Here's how the part is built. I have some questions about the finished solid (model axes, mm). A direction names the side the tool comes from. Coordinates: 2 decimals unless noted, no trailing zeros. Write each loop counter-clockwise with the first axis right and the second up, starting at its lowest first coordinate (ties: lowest second). Pieces come first, ordered by that corner, then holes. Notation, with made-up numbers: M 83.5,-31 L 95.5,-31 A22 ccw 95.5,1 Z; hole C 60.5,-1.75 d2. An arc over 180 degrees is marked long. Use a Markdown table: item, result.
```python
from build123d import *

# Parameters (mm, degrees)
BOSS_EXTRUDE1_DEPTH = 16
SKETCH2_W           = 8.91
SKETCH2_H           = 2
CUT_EXTRUDE1_DEPTH  = 10.3
CUT_EXTRUDE2_DEPTH  = 14.5
CUT_EXTRUDE3_DEPTH  = 14.5
BOSS_EXTRUDE2_DEPTH = 8


with BuildPart() as part:
    # Sketch1 → Boss-Extrude1 (new body)
    with BuildSketch(Plane.XY.offset(-14.5)):
        with BuildLine():
            Line((-5.37, 4.89), (-5.37, 0.647359313))
            Line((-5.37, 0.647359313), (-4.258679656, 1.758679656))
            Line((-4.258679656, 1.758679656), (-0.707106781, -1.792893219))
            ThreePointArc((-0.707106781, -1.792893219), (0, -2.085786438), (0.707106781, -1.792893219))
            Line((0.707106781, -1.792893219), (3.54, 1.04))
            Line((3.54, 1.04), (3.54, 4.89))
            Line((3.54, 4.89), (-5.37, 4.89))
        make_face()
    extrude(amount=BOSS_EXTRUDE1_DEPTH)

    # Sketch2 → Cut-Extrude1 (cut)
    with BuildSketch(Plane.XY.offset(-14.5)):
        with Locations((-0.915, 3.89)):
            Rectangle(SKETCH2_W, SKETCH2_H)
    extrude(amount=CUT_EXTRUDE1_DEPTH, mode=Mode.SUBTRACT)

    # Sketch3 → Cut-Extrude2 (cut)
    with BuildSketch(Plane.XY):
        with BuildLine():
            Line((-2.64, 0.14), (-2.64, -5))
            Line((-2.64, -5), (2.64, -5))
            Line((2.64, -5), (2.64, 0.14))
            Line((2.64, 0.14), (2.567267895, 0.067267895))
            ThreePointArc((2.567267895, 0.067267895), (2.355135861, -0.020600071), (2.143003826, 0.067267895))
            Line((2.143003826, 0.067267895), (2.070271721, 0.14))
            ThreePointArc((2.070271721, 0.14), (1.898724344, 0.836941375), (1.5, 1.433745096))
            Line((1.5, 1.433745096), (1.5, 2.89))
            Line((1.5, 2.89), (-1.5, 2.89))
            Line((-1.5, 2.89), (-1.5, 1.433745096))
            ThreePointArc((-1.5, 1.433745096), (-1.898724344, 0.836941375), (-2.070271721, 0.14))
            Line((-2.070271721, 0.14), (-2.143003826, 0.067267895))
            ThreePointArc((-2.143003826, 0.067267895), (-2.355135861, -0.020600071), (-2.567267895, 0.067267895))
            Line((-2.567267895, 0.067267895), (-2.64, 0.14))
        make_face()
    extrude(amount=-CUT_EXTRUDE2_DEPTH, mode=Mode.SUBTRACT)

    # Sketch4 → Cut-Extrude3 (cut)
    with BuildSketch(Plane.XY):
        Polygon((-5.37, 0.647359313), (-3.127359313, 2.89), (-5.37, 2.89), align=None)
    extrude(amount=-CUT_EXTRUDE3_DEPTH, mode=Mode.SUBTRACT)

    # Sketch5 → Boss-Extrude2 (add)
    with BuildSketch(Plane.XY.offset(-6.5)):
        Polygon((-12.228935778, -1.968935778), (-10.107615434, -4.090256121), (-8.39288149, -2.375522177), (-7.897906743, -2.870496924), (-5.670520382, -0.643110563), (-6.165495129, -0.148135816), (-3.248679656, 2.768679656), (-5.37, 4.89), align=None)
    extrude(amount=BOSS_EXTRUDE2_DEPTH)

    # Sketch6 → Cut-Revolve1 (revolve, cut)
    with BuildSketch(Plane.XY.offset(-2.5), mode=Mode.PRIVATE) as cut_revolve1_sk:
        Polygon((-5.894974747, -2.676042559), (-6.955634919, -3.73670273), (-10.491168825, -0.201168825), (-9.430508653, 0.859491347), align=None)
    revolve(cut_revolve1_sk.sketch.rotate(Axis((-9.430508653, 0.859491347, -2.5), (0.7071067811865479, -0.7071067811865472, 0)), 180), axis=Axis((-9.430508653, 0.859491347, -2.5), (0.7071067811865479, -0.7071067811865472, 0)), mode=Mode.SUBTRACT)

    # Sketch7 → Revolve1 (revolve)
    with BuildSketch(Plane(origin=(0, 0, 0), x_dir=(0, 0, -1), z_dir=(1, 0, 0)), mode=Mode.PRIVATE) as revolve1_sk:
        with BuildLine():
            Line((1.5, 4.69), (-0.7, 4.69))
            Line((-0.7, 4.69), (-0.7, 4.89))
            Line((-0.7, 4.89), (-0.35, 4.89))
            ThreePointArc((-0.35, 4.89), (-0.632842712, 5.007157288), (-0.75, 5.29))
            Line((-0.75, 5.29), (-0.75, 5.470108292))
            ThreePointArc((-0.75, 5.470108292), (-0.700420617, 5.781075575), (-0.556598698, 6.061207725))
            ThreePointArc((-0.556598698, 6.061207725), (0.348255742, 6.809981308), (1.5, 7.04))
            Line((1.5, 7.04), (1.5, 4.69))
        make_face()
    revolve(revolve1_sk.sketch.rotate(Axis((0, 7.04, -1.5), (0, -1, 0)), 180), axis=Axis((0, 7.04, -1.5), (0, -1, 0)))


solid = part.part
```
1. Suppose I cut it at A-A on z = -9.75. Write out the boundary of the cut face in (x, y) (3 decimals), and give its area (3 significant figures).
Answers follow:
| item | result |
|---|---|
| outline | M -4.259,1.759 L -2.567,0.067 A0.3 ccw -2.143,0.067 L -2.07,0.14 A2.075 cw -1.5,1.434 L -1.5,2.89 L -3.127,2.89 Z; M 1.5,1.434 A2.075 cw 2.07,0.14 L 2.143,0.067 A0.3 ccw 2.567,0.067 L 3.54,1.04 L 3.54,2.89 L 1.5,2.89 Z |
| area | 9.99 mm2 |
2. Will these pins go through, and if not, where does the flat tip stop? pin 1 Ø4.5 at (x, y) = (-7.5, 2) entering from -Z; pin 2 Ø1.5 at (x, y) = (-1, -0.5) entering from -Z; pin 3 Ø1 at (x, y) = (-1.5, 4) entering from -Z.
Answers follow:
| item | result |
|---|---|
| pin 1 | stops at z = -6.5 |
| pin 2 | stops at z = 0 |
| pin 3 | stops at z = -4.2 |
3. I need wall thicknesses on probe 1 along X at (y, z) = (1.5, -3); probe 2 along X at (y, z) = (1.25, -4.5); probe 3 along Z at (x, y) = (-0.25, -0.5). Which ranges of each line are inside material? Lowest first, please.
Answers follow:
| item | result |
|---|---|
| probe 1 | x = -8.07 to -4.52, -4 to -1.5, 1.5 to 3.54 |
| probe 2 | x = -9.01 to -4.77, -3.75 to -1.66, 1.66 to 3.54 |
| probe 3 | z = 0 to 1.5 |
4. We'd pull the mould along Y, two halves only. Please class faces 1 (the face through (3, 2, -14.5)), 2 (the face through (-1.895, 0.846, -7.148)), 3 (the face through (-8.356, -0.675, -3.964)): +Y half, -Y half, draft (parallel to the pull), parting line (faces both ways), or undercut.
Answers follow:
| item | result |
|---|---|
| face 1 | draft |
| face 2 | -Y half |
| face 3 | undercut |
5. Which directions (+Z, -Z, +X, -X, +Y, -Y) give clear straight access to the entire face, cutting with the end or side of a thin tool? Please do faces 4 (the face through (1.5, 2, -7)), 5 (the face through (-2, 2.89, -9)), 6 (the face through (-3.2, 0.7, -6.4)).
Answers follow:
| item | result |
|---|---|
| face 4 | -Z, -Y |
| face 5 | -Z, +X, +Y |
| face 6 | +Z, -Z, -Y |
6. Suppose I cut it at B-B on z = -2.75. State how many separate pieces and enclosed holes the cut face has, and give its area (3 significant figures).
Answers follow:
| item | result |
|---|---|
| separate pieces | 2 |
| enclosed holes | 1 |
| area | 52.0 mm2 |
